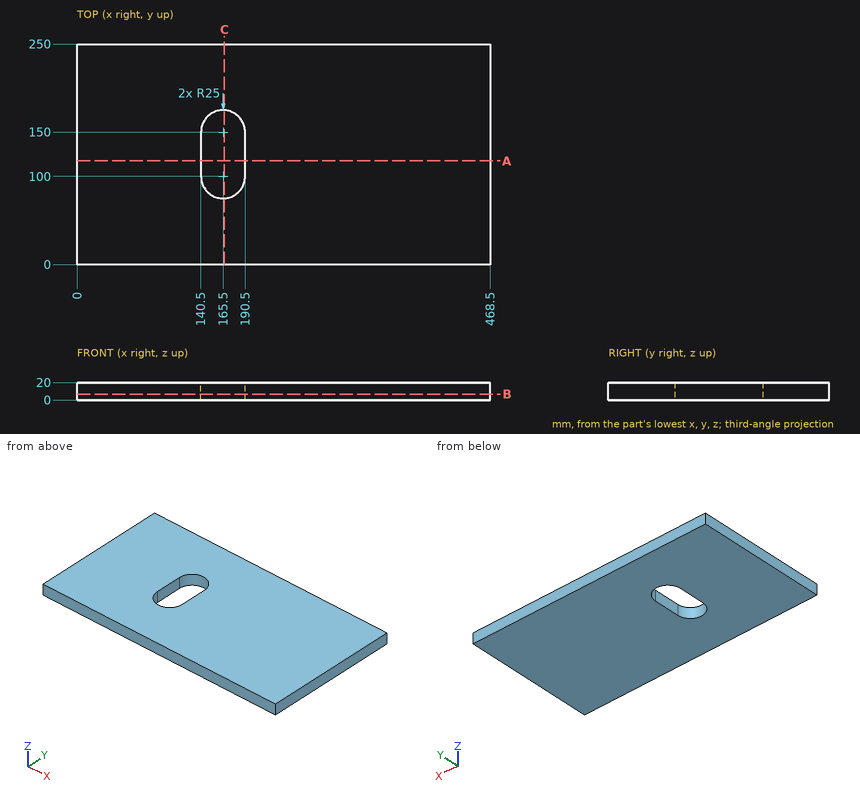
Geometry: see drawing. Coordinates: mm, zero at the bounding-box minimum. Give positions to 0.01 mm unless a question says otherwise; leave off trailing zeros. Loops run counter-clockwise (first coordinate to the right, second up) from the corner with the lowest first, then second, coordinate; pieces in that order, holes last. Notation, with made-up numbers: (-32.5, -35) -> (-10.5, -35) arc R20 ccw to (-10.5, -29) -> close; hole circle Ø3 at (69, 63.25). An arc over 180 degrees is marked (long way). Answer as a JSON object with one key per item and string values. Group by question number.
Item 1: Cut plane B-B, the plane z = 7. Return the cut outline in (x, y).
Item 2: Cut plane C-C, the plane x = 167. Return the cut outline in (y, z) (1 decimal).
Item 3: Line query: probe 1 along X at (y, z) = (149, 7.5); probe 2 along X at (y, z) = (92, 12.75) (1 decimal); probe 3 along Y at (x, z) = (180.5, 4). Output: solid intervals per line, ascending.
Item 4: Cut plane A-A, the plane y = 117.5. Return the cut outline in (x, z), and give its area (3 significant figures).
Checks:
{
 "1": {"outline": "(0, 0) -> (468.5, 0) -> (468.5, 250) -> (0, 250) -> close; hole (140.5, 100) arc R25 ccw to (190.5, 100) -> (190.5, 150) arc R25 ccw to (140.5, 150) -> close"},
 "2": {"outline": "(0, 0) -> (75, 0) -> (75, 20) -> (0, 20) -> close; (175, 0) -> (250, 0) -> (250, 20) -> (175, 20) -> close"},
 "3": {"probe 1": "x = 0 to 140.5, 190.5 to 468.5", "probe 2": "x = 0 to 141.8, 189.2 to 468.5", "probe 3": "y = 0 to 80, 170 to 250"},
 "4": {"outline": "(0, 0) -> (140.5, 0) -> (140.5, 20) -> (0, 20) -> close; (190.5, 0) -> (468.5, 0) -> (468.5, 20) -> (190.5, 20) -> close", "area": "8,370 mm²"}
}
